Job drawing, mm, ordinate dimensions from the low corner. One solid piece. A direction names the side the tool comes from. Give positions to 0.01 mm unless a question says otherwise; leave off trailing zeros. Loops run counter-clockwise (first coordinate to the right, second up) from the corner with the lowest first, then second, coordinate; pieces in that order, holes last.
Item 1: Mould opens along Y. For the marked faces 1, 2, 3 and 4 say: released by +Y, released by -Y, zero draft, split by the parting line, or undercut.
Item 2: Saw through at B-B on x = 7.25. Give the cut face in (y, z).
Item 3: Saw through at A-A on y = 35. Give the number of separate pieces and of enclosed holes in the cut face, plus the area to 3 significant figures.
Item 4: Which spindle directions (+Z, -Z, +X, -X, +Y, -Y) get a long thin tool onto all of the face, cutting with end or side? Do the marked faces 5, 6 and 7. Say none if no direction does.
Item 5: Saw through at D-D on x = 12. Give the cut face in (y, z), plus the area to 3 significant figures.
Item 6: Drop flat-ended pins along their axis: P1, Ø9, axis at y = 19.67, z = 35, coming from the -X side; P2, Ø10.5, axis at y = 35, z = 50.33, coming from the +X side; P3, Ø1.5, axis at x = 5.5, z = 46, coming from the -Y side (1 decimal). Give the stop position or say it passes through.
Item 7: Probe probe 1 along Y at (x, z) = (7.75, 33.5); probe 2 along X at (y, z) = (55, 27.5). List the from-to ranges inside material, lowest first.
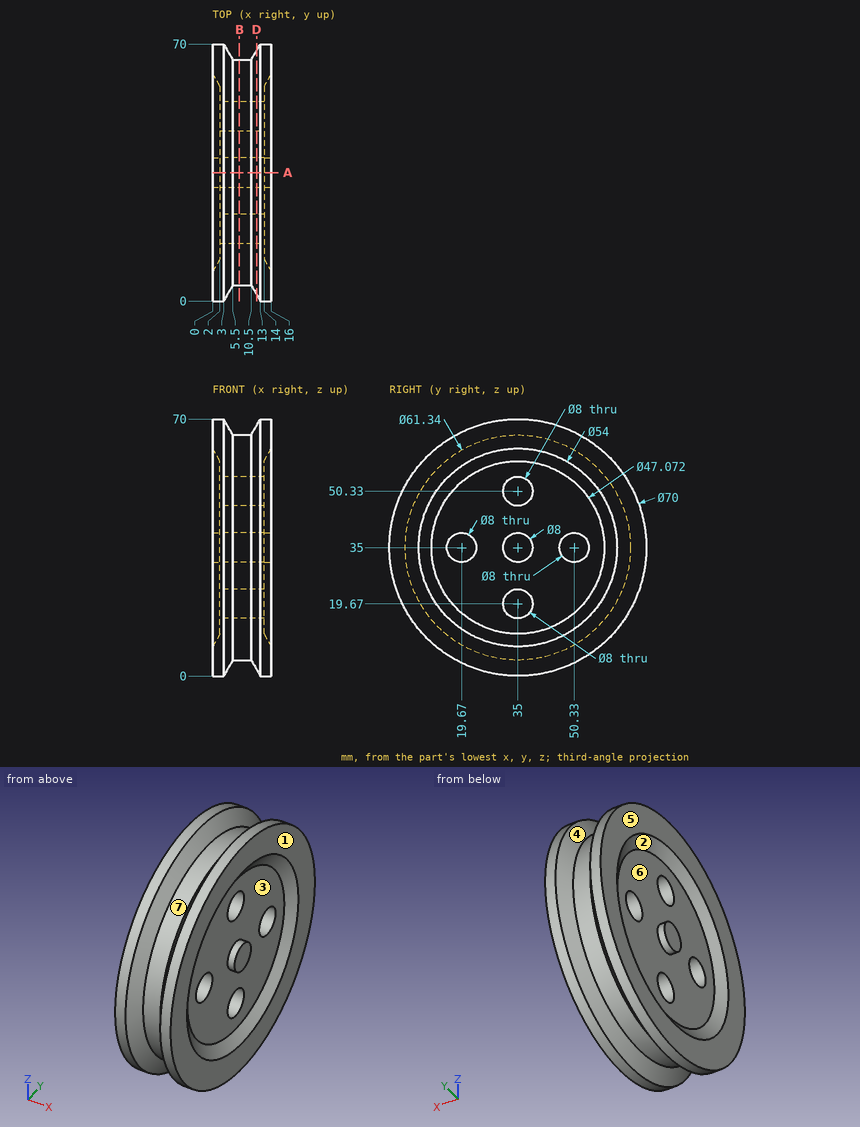
Results below:
1. face 1: zero draft
1. face 2: undercut
1. face 3: undercut
1. face 4: split by the parting line
2. outline: circle Ø61.34 at (35, 35); hole circle Ø8 at (19.67, 35); hole circle Ø8 at (35, 19.67); hole circle Ø8 at (35, 50.33); hole circle Ø8 at (50.33, 35)
3. separate pieces: 3
3. enclosed holes: 0
3. area: 693 mm2
4. face 5: +Z, -Z, -X, +Y, -Y
4. face 6: -X
4. face 7: none
5. outline: circle Ø66.54 at (35, 35); hole circle Ø8 at (19.67, 35); hole circle Ø8 at (35, 19.67); hole circle Ø8 at (35, 50.33); hole circle Ø8 at (50.33, 35)
5. area: 3,280 mm2
6. P1: stops at x = 2
6. P2: stops at x = 14
6. P3: stops at y = 5
7. probe 1: y = 4.37 to 15.96, 23.38 to 46.62, 54.04 to 65.63
7. probe 2: x = 2 to 14
